Source: CAD feature listing. Evaluate the final solid. Frame: model axes, mm. A direction names the side the tool comes from. Give positions to 0.01 mm unless a question says otherwise; leave off trailing zeros. Loops run counter-clockwise (first coordinate to the right, second up) from the corner with the lowest first, then second, coordinate; pieces in that order, holes last.
```python
from build123d import *

# Parameters (mm, degrees)
SKETCH1_R           = 4
BOSS_EXTRUDE1_DEPTH = 10


with BuildPart() as part:
    # Sketch1 → Boss-Extrude1 (new body)
    with BuildSketch(Plane.XY):
        with BuildLine():
            Line((5.291502622, -6), (24.708497378, -6))
            ThreePointArc((24.708497378, -6), (38, 0), (24.708497378, 6))
            Line((24.708497378, 6), (5.291502622, 6))
            ThreePointArc((5.291502622, 6), (-8, 0), (5.291502622, -6))
        make_face()
        Circle(SKETCH1_R, mode=Mode.SUBTRACT)
        with Locations((30, 0)):
            Circle(SKETCH1_R, mode=Mode.SUBTRACT)
    extrude(amount=BOSS_EXTRUDE1_DEPTH)


solid = part.part
```
(1) First-contact query: pin 1 (1 mm diameter, centred on y = 3, z = 5.5, fed in from -X); pin 2 (3 mm diameter, centred on x = 23, z = 3.5, fed in from +Y); pin 3 (1 mm diameter, centred on y = -4.5, z = 7.5, fed in from -X); pin 4 (7 mm diameter, centred on x = 30, y = 0, fed in from -Z). Flat tips, straight axial feed; report the tip coordinate or a pass-through.
A:
pin 1: stops at x = -7.6
pin 2: stops at y = 6
pin 3: stops at x = -6.93
pin 4: passes through
(2) Section B-B, the plane z = 4. Return the cut outline in (x, y), then the cut area to 3 significant figures.
A:
outline: (5.29, -6) - (24.71, -6) arc R8 ccw (long way) to (24.71, 6) - (5.29, 6) arc R8 ccw (long way) to start; hole circle Ø8 at (0, 0); hole circle Ø8 at (30, 0)
area: 490 mm2
(3) Ray query, line 1 along X through (y, z) = (2.75, 3.5); line 2 along Y through (x, z) = (30, 5.25); line 3 along X through (y, z) = (1.75, 3). Return the intervals inside material, ascending.
A:
line 1: x = -7.51 to -2.9, 2.9 to 27.1, 32.9 to 37.51
line 2: y = -8 to -4, 4 to 8
line 3: x = -7.81 to -3.6, 3.6 to 26.4, 33.6 to 37.81
(4) Section C-C, the plane y = -3.5. Return the cut outline in (x, z), then the cut area to 3 significant figures.
A:
outline: (-7.19, 0) - (-1.94, 0) - (-1.94, 10) - (-7.19, 10) - close; (1.94, 0) - (28.06, 0) - (28.06, 10) - (1.94, 10) - close; (31.94, 0) - (37.19, 0) - (37.19, 10) - (31.94, 10) - close
area: 366 mm2
(5) Section D-D, the plane y = 6.75. Return the cut outline in (x, z).
A:
outline: (-4.29, 0) - (4.29, 0) - (4.29, 10) - (-4.29, 10) - close; (25.71, 0) - (34.29, 0) - (34.29, 10) - (25.71, 10) - close
(6) Section A-A, the plane x = 0. Return the cut outline in (y, z), then the cut area to 3 significant figures.
A:
outline: (-8, 0) - (-4, 0) - (-4, 10) - (-8, 10) - close; (4, 0) - (8, 0) - (8, 10) - (4, 10) - close
area: 80.0 mm2
(7) Reachability of faces 1 (the flat face through (15, -6, 5)), 2 (the flat face through (15, 0, 10)), 3 (the flat face through (15, 6, 5)) from +Z, -Z, +X, -X, +Y, -Y: full face, straight path, thin tool, end or side. Return the list, or none.
A:
face 1: +Z, -Z, -Y
face 2: +Z, +X, -X, +Y, -Y
face 3: +Z, -Z, +Y
(8) Mould query, pull axis Y, two halves, no side actions, for faces 4 (the flat face through (15, 0, 0)), 5 (the cylindrical face through (26.8, -2.4, 4.9)), 6 (the cylindrical face through (-8, 0, 5)). Classes: pulls with the +Y half, pulls with the -Y half, needs draft (parallel to the pull), parting line crosses it, or undercut.
A:
face 4: needs draft
face 5: undercut
face 6: parting line crosses it
